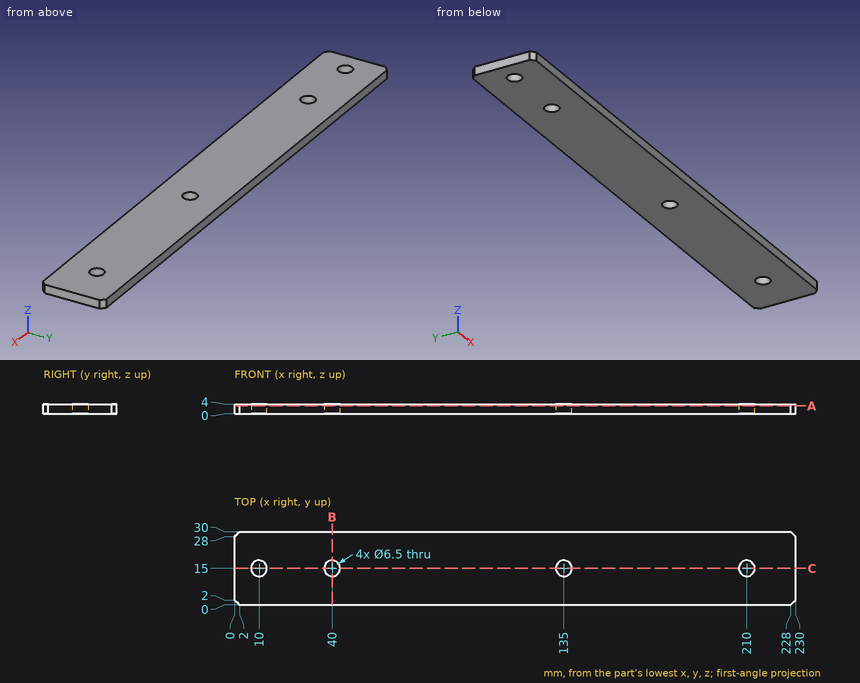
Drawing for the job (mm, zero at the part's lowest x, y, z). Round coordinates to 2 decimals unless told otherwise and drop trailing zeros. Order: outer loops, then holes, each group sorted by start corner. A loop starts at its lowest first (then second) coordinate and runs counter-clockwise, first axis right, second up.
Item 1: Saw through at A-A on z = 3.25. Write the cut outline in (x, y), then the cut area to 3 significant figures.
Item 2: Probe line 1 along Y through (x, z) = (40, 1.4); line 2 along X through (y, z) = (15.5, 3.5). List the from-to ranges inside material, lowest first.
Item 3: Saw through at C-C on y = 15. Write the cut outline in (x, z).
Item 4: Saw through at B-B on x = 40. Write the cut outline in (y, z).
Item 5: Pin check, flat tip, straight feed: pin 1 (8.5 mm diameter, centred on x = 135, y = 15, fed in from -Z). Stop position of the tip, or through.
Reported:
1. outline: (0, 2) - (2, 0) - (228, 0) - (230, 2) - (230, 28) - (228, 30) - (2, 30) - (0, 28) - close; hole circle Ø6.5 at (10, 15); hole circle Ø6.5 at (40, 15); hole circle Ø6.5 at (135, 15); hole circle Ø6.5 at (210, 15)
1. area: 6,760 mm2
2. line 1: y = 0 to 11.75, 18.25 to 30
2. line 2: x = 0 to 6.79, 13.21 to 36.79, 43.21 to 131.79, 138.21 to 206.79, 213.21 to 230
3. outline: (0, 0) - (6.75, 0) - (6.75, 4) - (0, 4) - close; (13.25, 0) - (36.75, 0) - (36.75, 4) - (13.25, 4) - close; (43.25, 0) - (131.75, 0) - (131.75, 4) - (43.25, 4) - close; (138.25, 0) - (206.75, 0) - (206.75, 4) - (138.25, 4) - close; (213.25, 0) - (230, 0) - (230, 4) - (213.25, 4) - close
4. outline: (0, 0) - (11.75, 0) - (11.75, 4) - (0, 4) - close; (18.25, 0) - (30, 0) - (30, 4) - (18.25, 4) - close
5. pin 1: stops at z = 0
